```python
from build123d import *

# Parameters (mm, degrees)
SKETCH_1_R               = 100
EXTRUDE_1_DEPTH          = 100
SKETCH_2_R               = 200
EXTRUDE_2_DEPTH          = 200
SKETCH_3_R               = 300
EXTRUDE_3_DEPTH          = 100
CUT_EXTRUDE_1_DEPTH      = 10
PATTERN_CIRCULAR_1_COUNT = 3
FILLET_1_R               = 50
SCALE_1_SCALE            = 0.1


with BuildPart() as part:
    # 草图1 → 凸台-拉伸1 (new body)
    with BuildSketch(Plane.XY):
        Circle(SKETCH_1_R)
    extrude(amount=EXTRUDE_1_DEPTH)

    # 草图2 → 凸台-拉伸2 (add)
    with BuildSketch(Plane.XY.offset(100)):
        Circle(SKETCH_2_R)
    extrude(amount=EXTRUDE_2_DEPTH)

    # 草图3 → 凸台-拉伸3 (add)
    with BuildSketch(Plane.XY.offset(300)):
        Circle(SKETCH_3_R)
    extrude(amount=EXTRUDE_3_DEPTH)

    # 草图4 → 切除-拉伸1 (cut)
    with BuildSketch(Plane.XY.offset(400)):
        with BuildLine():
            Line((-188.355536126, 50.469713795), (-198.014794389, 53.057904246))
            ThreePointArc((-198.014794389, 53.057904246), (-162.63743476, 124.796092947), (-102.5, 177.535207776))
            Line((-102.5, 177.535207776), (-105, 181.865334795))
            Line((-105, 181.865334795), (-51.763809021, 193.185165258))
            Line((-51.763809021, 193.185165258), (-95, 164.544826719))
            Line((-95, 164.544826719), (-97.5, 168.874953738))
            ThreePointArc((-97.5, 168.874953738), (-154.703901357, 118.708478657), (-188.355536126, 50.469713795))
        make_face()
    cut_extrude_1 = extrude(amount=-CUT_EXTRUDE_1_DEPTH, mode=Mode.SUBTRACT)

    # 阵列(圆周)1: 切除-拉伸1 ×3 about axis
    pattern_circular_1_axis = Axis((0, 0, 0), (0, 0, 1))
    for i in range(1, PATTERN_CIRCULAR_1_COUNT):
        add(cut_extrude_1.rotate(pattern_circular_1_axis, i * 360 / PATTERN_CIRCULAR_1_COUNT), mode=Mode.SUBTRACT)

    # 圆角1
    fillet_1_edges = [part.edges().sort_by_distance(p)[0] for p in [
        (-300, 0, 400),
    ]]
    fillet(fillet_1_edges, radius=FILLET_1_R)


with BuildPart() as part_1:
    # 缩放比例1: scaled about (0, 0, 264.382298041)
    add(part.part.scale(SCALE_1_SCALE).moved(Location((0, 0, 237.944068237))))


solid = part_1.part
```
Design review of the part built by this model. Coordinates are the model's own, in mm. A direction names the side the tool comes from. Coordinates: 2 decimals unless noted, no trailing zeros. Loops run counter-clockwise (first coordinate to the right, second up) from the corner with the lowest first, then second, coordinate; pieces in that order, holes last. Notation, with made-up numbers: (65, 31) - (110, 31) arc R20 ccw to (110, 65) - close; hole circle Ø2 at (9.25, 15.5). An arc over 180 degrees is marked (long way). Use CSV: the item, a comma, the result in double quotes. Start each with the question number.
1) Consider section A-A on x = 0. Write out the cut boundary in (y, z), then the cut area to 3 significant figures.
2) For pin 1 Ø1 at (x, z) = (-19, 257) entering from +Y; pin 2 Ø1.5 at (x, y) = (-10, -8) entering from -Z; pin 3 Ø1.5 at (y, z) = (16, 251) entering from +X; pin 4 Ø18 at (x, y) = (10, -10) entering from -Z, all flat-tipped, find the tip position at first contact; note any pin that passes through.
3) Wall thickness on L1, parallel to Z at x = 13, y = -8.5; L2, parallel to X at y = -4.5, z = 249.5; L3, parallel to X at y = -0.5, z = 272: over which ranges is each line inside the solid? List them lowest first. Write a range as from..to.
4) Consider section C-C on z = 270.5. Write out the cut boundary in (x, y), then the cut area to 3 significant figures.
5) The part is to be moulded in two halves that separate along X. For faces 4 (the flat face through (-14, 14, 276.944)), 5 (the cylindrical face through (-2.17, -9.76, 242.87)), 6 (the flat face through (20, -6, 267.944)), say which applies: +X half, -X half, draft (parallel to the pull), parting line (faces both ways), or undercut.
6) Consider section B-B on z = 242. Write out the cut boundary in (x, y).
7) Tool access review of faces 1 (the flat face through (0, 0, 277.944)), 2 (the flat face through (-5, 9, 247.944)), 3 (the cylindrical face through (-16.33, 12.39, 277.45)): name each direction out of +Z, -Z, +X, -X, +Y, -Y from which nothing blocks a thin tool from reaching the whole face with its end or side.
Geometry says:
1,outline,"(-30, 267.94) - (-20, 267.94) - (-20, 247.94) - (-10, 247.94) - (-10, 237.94) - (10, 237.94) - (10, 247.94) - (20, 247.94) - (20, 267.94) - (30, 267.94) - (30, 272.94) arc R5 ccw to (25, 277.94) - (-19.5, 277.94) - (-19.5, 276.94) - (-20.5, 276.94) - (-20.5, 277.94) - (-25, 277.94) arc R5 ccw to (-30, 272.94) - close"
1,area,"1,590 mm^2"
2,pin 1,"y = 7.6"
2,pin 2,"z = 247.94"
2,pin 3,"x = 12.94"
2,pin 4,"z = 237.94"
3,L1,"247.94..277.94"
3,L2,"-19.49..19.49"
3,L3,"-30..30"
4,outline,"circle Ø60 at (0, 0)"
4,area,"2,830 mm^2"
5,face 4,"undercut"
5,face 5,"parting line"
5,face 6,"draft"
6,outline,"circle Ø20 at (0, 0)"
7,face 1,"+Z, +X, -X, +Y, -Y"
7,face 2,"-Z"
7,face 3,"+Z"
